Can you work these out from the model? Positions are in its coordinate system, mm. Face numbers are marked on the shaded views. Round coordinates to 2 decimals unless told otherwise and drop trailing zeros. Write each loop counter-clockwise with the first axis right and the second up, starting at its lowest first coordinate (ties: lowest second). Pieces come first, ordered by that corner, then holes.
Q1. Please list where these lines run through material, in increasing order: line 1 along Y through (x, z) = (0, 5.5); line 2 along Y through (x, z) = (-20, 7.25); line 3 along X through (y, z) = (5, 15.75).
Q2. We'd pull the mould along Y, two halves only. Please class the marked faces 1, 2 and 3: +Y half, -Y half, draft (parallel to the pull), parting line (faces both ways), or undercut.
Q3. If we section it at A-A (x = 0): Please give me the cut outline in (y, z), plus the area to 3 significant figures.
Q4. If we section it at C-C (z = 3.5): Please give me the cut outline in (x, y), plus the area to 3 significant figures.
Q5. I'm going to push flat-ended pins straight in: pin 1 Ø4 at (x, y) = (-19.5, 13) entering from -Z; pin 2 Ø6 at (x, z) = (13.5, 17) entering from +Y; pin 3 Ø2 at (y, z) = (10, 6) entering from -X; pin 4 Ø8 at (x, z) = (-12, 10) entering from -Y. Where does each tip first touch, or does it pass through?
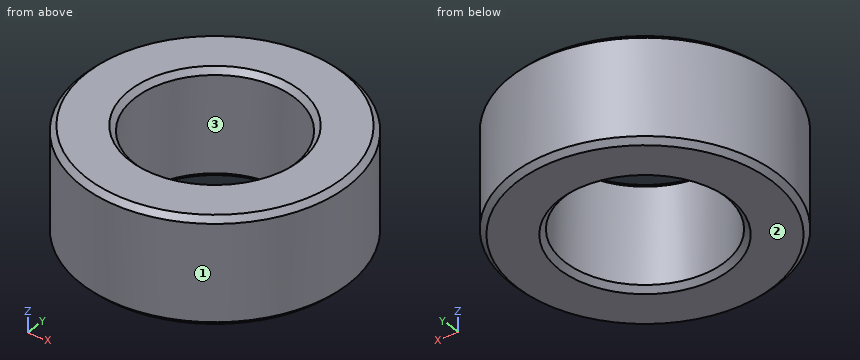
from build123d import *

# Parameters (mm, degrees)
SKETCH1_R           = 25
SKETCH1_R_2         = 15
BOSS_EXTRUDE1_DEPTH = 20
CHAMFER1_SIZE       = 1


with BuildPart() as part:
    # Sketch1 → Boss-Extrude1 (new body)
    with BuildSketch(Plane.XY):
        Circle(SKETCH1_R)
        Circle(SKETCH1_R_2, mode=Mode.SUBTRACT)
    extrude(amount=BOSS_EXTRUDE1_DEPTH)

    # Chamfer1
    chamfer1_edges = [part.edges().sort_by_distance(p)[0] for p in [
        (-25, 0, 0),
        (-25, 0, 20),
        (-15, 0, 0),
        (-15, 0, 20),
    ]]
    chamfer(chamfer1_edges, length=CHAMFER1_SIZE)


solid = part.part
A:
1. line 1: y = -25 to -15, 15 to 25
1. line 2: y = -15 to 15
1. line 3: x = -24.49 to -14.14, 14.14 to 24.49
2. face 1: parting line
2. face 2: draft
2. face 3: undercut
3. outline: (-25, 1) - (-24, 0) - (-16, 0) - (-15, 1) - (-15, 19) - (-16, 20) - (-24, 20) - (-25, 19) - close; (15, 1) - (16, 0) - (24, 0) - (25, 1) - (25, 19) - (24, 20) - (16, 20) - (15, 19) - close
3. area: 396 mm2
4. outline: circle Ø50 at (0, 0); hole circle Ø30 at (0, 0)
4. area: 1,260 mm2
5. pin 1: stops at z = 0
5. pin 2: stops at y = 22.69
5. pin 3: stops at x = -23.32
5. pin 4: stops at y = -23.69
